Build history of the part. All positions in model axes, mm. Give positions to 0.01 mm unless a question says otherwise; leave off trailing zeros. Write each loop counter-clockwise with the first axis right and the second up, starting at its lowest first coordinate (ties: lowest second). Pieces come first, ordered by that corner, then holes. Notation, with made-up numbers: (41.25, 11.25) -> (97.25, 11.25) arc R24 ccw to (97.25, 39.25) -> close; hole circle Ø4 at (-29, 71.25). An arc over 180 degrees is marked (long way). One line per question, with ' | ' between items. Start each with the question number.
(1) Band-saw the part on D-D, the plane x = 20.5. Give the cut face in (y, z), and give its area (3 significant figures).
(2) Pin check, flat tips, straight feed: P1, Ø3, axis at x = 20, z = 4.5, coming from the +Y side; P2, Ø2, axis at y = 16.5, z = 2, coming from the +X side; P3, Ø11.5, axis at x = -18.52, y = 21.38, coming from the -Z side. Stop position of each tip, or through.
(3) Band-saw the part on C-C, the plane y = -41.5. Give the cut face in (x, z), and give its area (3 significant figures).
(4) Drill centre lines: probe 1 along X at (y, z) = (26, 2.4); probe 2 along Y at (x, z) = (12, 2); probe 3 along X at (y, z) = (23, 2.15). Where is each one in solid material? Low to high. Write a range as from..to.
(5) Band-saw the part on A-A, the plane x = -19.5. Give the cut face in (y, z), and give its area (3 significant figures).
(6) Band-saw the part on B-B, the plane z = 4.9. Give the cut face in (x, y).
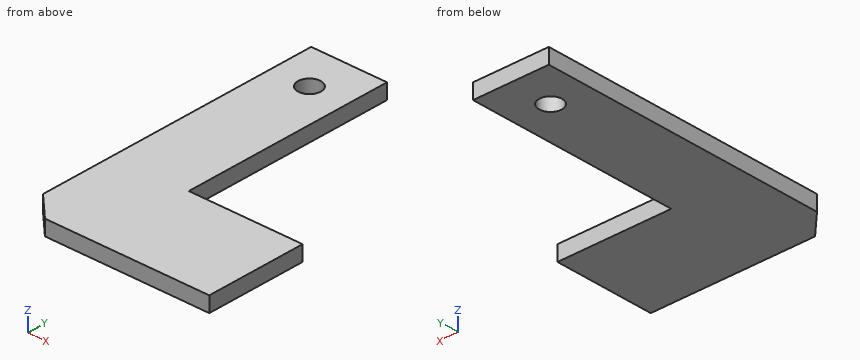
from build123d import *

# Parameters (mm, degrees)
BOSS_EXTRUDE1_DEPTH = 6
CUT_EXTRUDE1_REACH  = 98.228
SKETCH2_R           = 4.5
CHAMFER1_SIZE       = 10


with BuildPart() as part:
    # Sketch1 → Boss-Extrude1 (new body)
    with BuildSketch(Plane.XY):
        Polygon((-33.521587555, -86.6224812), (-33.521587555, 38.3775188), (-3.521587555, 38.3775188), (-3.521587555, -46.6224812), (41.478412445, -46.6224812), (41.478412445, -86.6224812), align=None)
    extrude(amount=BOSS_EXTRUDE1_DEPTH)

    # Sketch2 → Cut-Extrude1 (cut, up to next)
    with BuildSketch(Plane.XY.offset(6), mode=Mode.PRIVATE) as cut_extrude1_sk1:
        with Locations((-18.521587555, 21.3775188)):
            Circle(SKETCH2_R)
    cut_extrude1_tool1 = extrude(cut_extrude1_sk1.sketch, amount=-CUT_EXTRUDE1_REACH, mode=Mode.PRIVATE) & part.part
    add(cut_extrude1_tool1.solids().sort_by_distance((-18.521588, 21.377519, 6))[0], mode=Mode.SUBTRACT)

    # Chamfer1
    chamfer1_edges = [part.edges().sort_by_distance(p)[0] for p in [
        (-33.521587555, -86.6224812, 3),
    ]]
    chamfer(chamfer1_edges, length=CHAMFER1_SIZE)


solid = part.part
Results:
1) outline: (-86.62, 0) -> (-46.62, 0) -> (-46.62, 6) -> (-86.62, 6) -> close | area: 240 mm²
2) P1: stops at y = -46.62 | P2: stops at x = -3.52 | P3: stops at z = 0
3) outline: (-33.52, 0) -> (-3.52, 0) -> (-3.52, 6) -> (-33.52, 6) -> close | area: 180 mm²
4) probe 1: x = -33.52..-3.52 | probe 2: y = -86.62..-46.62 | probe 3: x = -33.52..-22.72, -14.32..-3.52
5) outline: (-86.62, 0) -> (16.99, 0) -> (16.99, 6) -> (-86.62, 6) -> close; (25.77, 0) -> (38.38, 0) -> (38.38, 6) -> (25.77, 6) -> close | area: 697 mm²
6) outline: (-33.52, -76.62) -> (-23.52, -86.62) -> (41.48, -86.62) -> (41.48, -46.62) -> (-3.52, -46.62) -> (-3.52, 38.38) -> (-33.52, 38.38) -> close; hole circle Ø9 at (-18.52, 21.38)
